```python
from build123d import *

# Parameters (mm, degrees)
SKETCH1_W           = 410
SKETCH1_H           = 410
BOSS_EXTRUDE1_DEPTH = 18
SKETCH2_R           = 11
CUT_EXTRUDE1_DEPTH  = 18


with BuildPart() as part:
    # Sketch1 → Boss-Extrude1 (new body)
    with BuildSketch(Plane.XY):
        Rectangle(SKETCH1_W, SKETCH1_H)
    extrude(amount=BOSS_EXTRUDE1_DEPTH)

    # Sketch2 → Cut-Extrude1 (cut)
    with BuildSketch(Plane.XY.offset(18)):
        with Locations((-165, 165)):
            Circle(SKETCH2_R)
        with Locations((165, 165)):
            Circle(SKETCH2_R)
        with Locations((165, -165)):
            Circle(SKETCH2_R)
        with Locations((-165, -165)):
            Circle(SKETCH2_R)
        with Locations((-165, 55)):
            Circle(SKETCH2_R)
        with Locations((-165, -55)):
            Circle(SKETCH2_R)
        with Locations((-55, 165)):
            Circle(SKETCH2_R)
        with Locations((55, 165)):
            Circle(SKETCH2_R)
        with Locations((165, 55)):
            Circle(SKETCH2_R)
        with Locations((165, -55)):
            Circle(SKETCH2_R)
        with Locations((-55, -165)):
            Circle(SKETCH2_R)
        with Locations((55, -165)):
            Circle(SKETCH2_R)
    extrude(amount=-CUT_EXTRUDE1_DEPTH, mode=Mode.SUBTRACT)


solid = part.part
```
Part model, mm, in its own coordinate system. Round coordinates to 2 decimals unless told otherwise and drop trailing zeros. Order: outer loops, then holes, each group sorted by start corner. A loop starts at its lowest first (then second) coordinate and runs counter-clockwise, first axis right, second up. Notation, with made-up numbers: M 44,-24.75 L 78,-24.75 A24 cw 78,-3.75 Z; hole C -5.5,62 d10. An arc over 180 degrees is marked long. Put each result on its own line as item: value. Start each with the question number.
1. Two-plate mould, pull along X, no slides. Class faces 1 (the face through (-3, 3, 0)), 2 (the face through (205, -3, 9)), 3 (the face through (-205, -3, 9)), 4 (the face through (154, 55, 9)): +X half, -X half, draft (parallel to the pull), parting line (faces both ways), or undercut.
2. Drill centre lines: probe 1 along Y at (x, z) = (-165, 13.5); probe 2 along X at (y, z) = (172.5, 4.25). Where is each one in solid material? Low to high. Write a range as [from, to].
3. Slice it at D-D on x = -55. List the corners of the cut face in (y, z).
4. Slice it at A-A on y = 165. List the corners of the cut face in (x, z).
5. Slice it at C-C on z = 12.75. State how many separate pieces and enclosed holes the cut face has, then the cut area to 3 significant figures.
6. Drop a flat-ended pin along its axis: pin 1 (17.5 mm diameter, centred on x = -55, y = -165, fed in from -Z). Give the stop position or say it passes through.
Findings:
1. face 1: draft
1. face 2: +X half
1. face 3: -X half
1. face 4: undercut
2. probe 1: [-205, -176], [-154, -66], [-44, 44], [66, 154], [176, 205]
2. probe 2: [-205, -173.05], [-156.95, -63.05], [-46.95, 46.95], [63.05, 156.95], [173.05, 205]
3. outline: M -205,0 L -176,0 L -176,18 L -205,18 Z; M -154,0 L 154,0 L 154,18 L -154,18 Z; M 176,0 L 205,0 L 205,18 L 176,18 Z
4. outline: M -205,0 L -176,0 L -176,18 L -205,18 Z; M -154,0 L -66,0 L -66,18 L -154,18 Z; M -44,0 L 44,0 L 44,18 L -44,18 Z; M 66,0 L 154,0 L 154,18 L 66,18 Z; M 176,0 L 205,0 L 205,18 L 176,18 Z
5. separate pieces: 1
5. enclosed holes: 12
5. area: 164,000 mm2
6. pin 1: through
